CAD build for the part. Positions are in the model's coordinates, mm. Face numbers are marked on the shaded views. A direction names the side the tool comes from. Coordinates: 2 decimals unless noted, no trailing zeros. Order: outer loops, then holes, each group sorted by start corner. A loop starts at its lowest first (then second) coordinate and runs counter-clockwise, first axis right, second up. Notation, with made-up numbers: M -25.75,5 L 26.25,5 A14 ccw 26.25,19 Z; hole C -21.75,88 d10. An arc over 180 degrees is marked long. Write item = value, one per line.
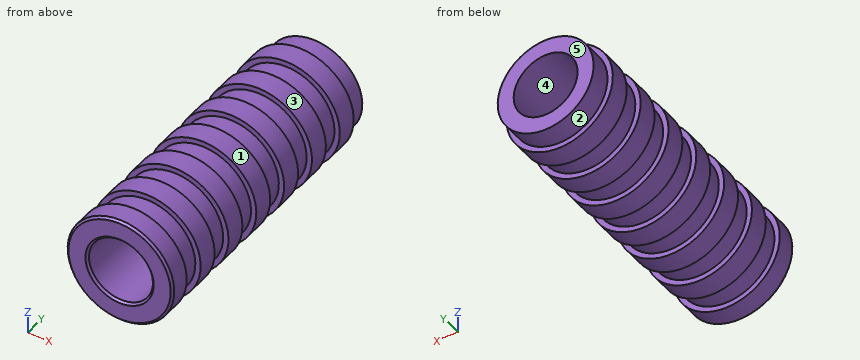
from build123d import *


with BuildPart() as part:
    # 草图1 → 旋转1 (revolve)
    with BuildSketch(Plane(origin=(0, 0, 0), x_dir=(-1, 0, 0), z_dir=(0, 0, -1)), mode=Mode.PRIVATE) as revolve_1_sk:
        Polygon((-22.5, -220), (-25, -220), (-25, -230), (-22.5, -230), (-22.5, -240), (-25, -240), (-25, -250), (-22.5, -250), (-22.5, -260), (-25, -260), (-25, -270), (-22.5, -270), (-22.5, -280), (-25, -280), (-25, -289), (-24, -290), (-16, -290), (-15, -289), (-15, -150), (-22.5, -150), (-22.5, -160), (-25, -160), (-25, -170), (-22.5, -170), (-22.5, -180), (-25, -180), (-25, -190), (-22.5, -190), (-22.5, -200), (-25, -200), (-25, -210), (-22.5, -210), align=None)
    revolve(revolve_1_sk.sketch.rotate(Axis((0, -290, 0), (0, 1, 0)), 270), axis=Axis((0, -290, 0), (0, 1, 0)))


solid = part.part
(1) Slice it at A-A, the plane y = -274.5. Write the cut outline in (x, z), then the cut area to 3 significant figures.
Evaluation:
outline = C 0,0 d45; hole C 0,0 d30
area = 884 mm²
(2) Pull direction X, two halves, no side cores. Call the marked faces 3, 4 and 5: +X half, -X half, draft (parallel to the pull), parting line (faces both ways), or undercut.
Evaluation:
face_3 = parting line
face_4 = undercut
face_5 = draft
(3) Tool access for the marked faces 1 and 2: list every direction of +Z, -Z, +X, -X, +Y, -Y with a clear straight run to the whole face (end or side of a thin tool).
Evaluation:
face_1 = +Y, -Y
face_2 = +Y
(4) Slice it at B-B, the plane y = -207.5. Write the cut outline in (x, z).
Evaluation:
outline = C 0,0 d50; hole C 0,0 d30
(5) Wall check: line 1 (X direction, y = -249, z = 0); line 2 (X direction, y = -219, z = 0); line 3 (Z direction, x = 5, y = -171.5). Give the ranges that are in metal, low to high. Write a range as from..to.
Evaluation:
line_1 = -25..-15, 15..25
line_2 = -22.5..-15, 15..22.5
line_3 = -21.94..-14.14, 14.14..21.94
(6) Pin check, flat tips, straight feed: pin 1 Ø6 at (y, z) = (-259, 7) entering from +X; pin 2 Ø10 at (x, y) = (-18.5, -265.5) entering from +Z; pin 3 Ø1.5 at (y, z) = (-235, 7) entering from -X; pin 4 Ø15 at (x, z) = (-5, -2.5) entering from +Y. Stop position of each tip, or through.
Evaluation:
pin_1 = 24.65
pin_2 = 21.04
pin_3 = -21.61
pin_4 = through
